Work out the finished part from the listing and answer in its coordinate system (mm). A direction names the side the tool comes from. Round coordinates to 2 decimals unless told otherwise and drop trailing zeros. Order: outer loops, then holes, each group sorted by start corner. A loop starts at its lowest first (then second) coordinate and runs counter-clockwise, first axis right, second up. Notation, with made-up numbers: (36, 64.5) - (61, 64.5) arc R22 ccw to (61, 93.5) - close; hole circle Ø6 at (-3, 32.25). An arc over 180 degrees is marked (long way). Answer in a Markdown table with one row per item.
from build123d import *

# Parameters (mm, degrees)
SKETCH_1_R          = 5
SKETCH_1_R_2        = 1.6
EXTRUDE_1_DEPTH     = 2
SKETCH_6_W          = 51.8
SKETCH_6_H          = 7
CUT_EXTRUDE_4_DEPTH = 63.659795723
FILLET_5_R          = 2
FILLET_6_R          = 2


with BuildPart() as part:
    # 草图1 → 凸台-拉伸1 (new body)
    with BuildSketch(Plane.XY):
        with BuildLine():
            Line((-26.3, -32.06084855), (-26.3, -46))
            Line((-26.3, -46), (42.5, -46))
            Line((42.5, -46), (42.5, -31.867732913))
            Line((42.5, -31.867732913), (6.12172987, 5.896984263))
            ThreePointArc((6.12172987, 5.896984263), (-1.211932074, 8.413157591), (-7.537237585, 3.929382851))
            Line((-7.537237585, 3.929382851), (-26.3, -32.06084855))
        make_face()
        Circle(SKETCH_1_R, mode=Mode.SUBTRACT)
        with Locations((-22.8, -34)):
            Circle(SKETCH_1_R_2, mode=Mode.SUBTRACT)
        with Locations((-22.8, -42)):
            Circle(SKETCH_1_R_2, mode=Mode.SUBTRACT)
        with Locations(Location((39, -42, 0), (0, 0, 180))):
            Circle(SKETCH_1_R_2, mode=Mode.SUBTRACT)
        with Locations(Location((39, -34, 0), (0, 0, 180))):
            Circle(SKETCH_1_R_2, mode=Mode.SUBTRACT)
    extrude(amount=EXTRUDE_1_DEPTH)

    # 草图6 → 切除-拉伸4 (cut, through all)
    with BuildSketch(Plane.XY.offset(2)):
        with BuildLine():
            Line((-7.552516715, -7.997467804), (-18.501752281, -29))
            Line((-18.501752281, -29), (1.7, -29))
            Line((1.7, -29), (-1.253662685, -10.928326948))
            ThreePointArc((-1.253662685, -10.928326948), (-4.640547676, -9.973230032), (-7.552516715, -7.997467804))
        make_face()
        with BuildLine():
            Line((4.667768527, -9.960518911), (7.779611281, -29))
            Line((7.779611281, -29), (32.100819179, -29))
            Line((32.100819179, -29), (9.502706469, -5.540629004))
            ThreePointArc((9.502706469, -5.540629004), (7.421889726, -8.118839381), (4.667768527, -9.960518911))
        make_face()
        with Locations((8.1, -37.5)):
            Rectangle(SKETCH_6_W, SKETCH_6_H)
    extrude(amount=-CUT_EXTRUDE_4_DEPTH, mode=Mode.SUBTRACT)

    # 圆角5
    fillet_5_edges = [part.edges().sort_by_distance(p)[0] for p in [
        (-17.8, -41, 1),
        (-17.8, -34, 1),
        (34, -34, 1),
        (34, -41, 1),
        (4.667768527, -9.960518911, 1),
        (9.502706469, -5.540629004, 1),
        (32.100819179, -29, 1),
        (7.779611281, -29, 1),
        (-7.552516715, -7.997467804, 1),
        (-1.253662685, -10.928326948, 1),
        (1.7, -29, 1),
        (-18.501752281, -29, 1),
    ]]
    fillet(fillet_5_edges, radius=FILLET_5_R)

    # 圆角6
    fillet_6_edges = [part.edges().sort_by_distance(p)[0] for p in [
        (42.5, -31.867732913, 1),
        (42.5, -46, 1),
        (-26.3, -46, 1),
        (-26.3, -32.06084855, 1),
    ]]
    fillet(fillet_6_edges, radius=FILLET_6_R)


solid = part.part
1) Find section D-D, the plane x = 35. Give the vertices of the cut face in (y, z), then the cut area to 3 significant figures.
Filled in:
| item | result |
|---|---|
| outline | (-46, 0) - (-24.08, 0) - (-24.08, 2) - (-46, 2) - close |
| area | 43.8 mm^2 |
2) Which of the six approach directions +Z, -Z, +X, -X, +Y, -Y give full straight-line access (tool end or side, diameter ignored) to faces 1 (the face through (-17.2, -34.57, 0.99)), 2 (the face through (42.5, -38, 1))?
Filled in:
| item | result |
|---|---|
| face 1 | +Z, -Z |
| face 2 | +Z, -Z, +X, +Y, -Y |
3) Find section B-B, the plane x = 20. Give the vertices of the cut face in (y, z), then the cut area to 3 significant figures.
Filled in:
| item | result |
|---|---|
| outline | (-46, 0) - (-41, 0) - (-41, 2) - (-46, 2) - close; (-34, 0) - (-29, 0) - (-29, 2) - (-34, 2) - close; (-16.44, 0) - (-8.51, 0) - (-8.51, 2) - (-16.44, 2) - close |
| area | 35.9 mm^2 |
4) Find section C-C, the plane z = 0.85. Give the number of separate pieces and of enclosed holes in the cut face, then the cut area to 3 significant figures.
Filled in:
| item | result |
|---|---|
| separate pieces | 1 |
| enclosed holes | 8 |
| area | 1,470 mm^2 |
5) The mould has two halves that part along X. Classify faces 3 (the face through (42.36, -31.94, 1.01)), 4 (the face through (8, -46, 1)), 5 (the face through (-17.8, -38, 1)), 6 (the face through (-22.06, -43.42, 0.99)): released by +X, released by -X, zero draft, split by the parting line, or undercut.
Filled in:
| item | result |
|---|---|
| face 3 | released by +X |
| face 4 | zero draft |
| face 5 | undercut |
| face 6 | undercut |
6) Find section A-A, the plane y = -42. Give the vertices of the cut face in (x, z), then the cut area to 3 significant figures.
Filled in:
| item | result |
|---|---|
| outline | (-26.3, 0) - (-24.4, 0) - (-24.4, 2) - (-26.3, 2) - close; (-21.2, 0) - (37.4, 0) - (37.4, 2) - (-21.2, 2) - close; (40.6, 0) - (42.5, 0) - (42.5, 2) - (40.6, 2) - close |
| area | 125 mm^2 |
7) This flat-tipped pin is pushed along its axis until it touches: pin 1 (0.6 mm diameter, centred on x = -0.5, z = 0.5, fed in from +Y). Where does it stop, or does it pass through?
Filled in:
| item | result |
|---|---|
| pin 1 | stops at y = 8.5 |
8) Find the intervals of material crossed by probe 1 along X at (y, z) = (-38, 0.85); probe 2 along Y at (x, z) = (11.5, 1.75); probe 3 along X at (y, z) = (-13, 1.4), in increasing order. Write a range as from..to.
Filled in:
| item | result |
|---|---|
| probe 1 | x = -26.3..-17.8, 34..42.5 |
| probe 2 | y = -46..-41, -34..-29, -7.61..0.31 |
| probe 3 | x = -16.36..-10.16, -0.92..5.16, 16.69..24.32 |
